Source: CAD feature listing. Evaluate the final solid. Frame: model axes, mm. A direction names the side the tool comes from. Give positions to 0.01 mm unless a question says otherwise; leave off trailing zeros. Order: outer loops, then holes, each group sorted by start corner. A loop starts at its lowest first (then second) coordinate and runs counter-clockwise, first axis right, second up. Notation, with made-up numbers: M 58.25,44.5 L 103.25,44.5 A9 ccw 103.25,57.5 Z; hole C 65,-35.5 d9. An arc over 180 degrees is marked long. Answer as a JSON object with one key per item and string values. Group by question number.
1. Section query A-A (y = -45). Output: boundary loops of the cut face in (x, z).
2. Pull-direction query (X, two-part tool) for faces 3 (the flat face through (-12.5, -1, 10)), 4 (the flat face through (-1.4, -49.2, 10)), 5 (the cylindrical face through (1.409, -51.345, 4.93)), 6 (the flat face through (-6, 1, 20)); classes: +X half, -X half, draft (parallel to the pull), parting line (faces both ways), or undercut.
3. Pin query (flat end, axial travel): P1, Ø6.5, axis at x = 1, y = -46.5, coming from the -Z side. Return the tip coordinate at first contact, or that it passes through.
4. Set-up query: faces 1 (the cylindrical face through (1.409, 38.655, 4.93)), 2 (the flat face through (-6, 1, 0)). Return all of +Z, -Z, +X, -X, +Y, -Y with unobstructed straight access to the full face (end or side cutting, diameter ignored); none if empty.
5. Section query B-B (x = 0). Output: boundary loops of the cut face in (y, z).
6. Section query C-C (z = 15.5). Output: boundary loops of the cut face in (x, y).
7. Section query D-D (y = 0). Output: boundary loops of the cut face in (x, z), plus the area to 3 significant figures.
8. Material intervals for L1, parallel to Y at x = 0, z = 5.5; L2, parallel to Y at x = 0, z = 15.75; L3, parallel to Z at x = -4.75, y = -48, sorted ascending. Write a range as [from, to].
from build123d import *

# Parameters (mm, degrees)
SKETCH1_W                   = 25
SKETCH1_H                   = 110
BOSS_EXTRUDE1_DEPTH         = 20
SKETCH3_R                   = 4.25
CUT_EXTRUDE1_DEPTH          = 30
SKETCH5_R                   = 6.5
CUT_EXTRUDE3_DEPTH          = 10
M12X1_25_TAPPED_HOLE1_D     = 10.5
M12X1_25_TAPPED_HOLE1_DEPTH = 30.25
M12X1_25_TAPPED_HOLE1_TIP   = 3.15451825


with BuildPart() as part:
    # Sketch1 → Boss-Extrude1 (new body)
    with BuildSketch(Plane.XY):
        Rectangle(SKETCH1_W, SKETCH1_H)
    extrude(amount=BOSS_EXTRUDE1_DEPTH)

    # Sketch3 → Cut-Extrude1 (cut)
    with BuildSketch(Plane.XY.offset(20)):
        with Locations((0, 45)):
            Circle(SKETCH3_R)
        with Locations((0, -45)):
            Circle(SKETCH3_R)
    extrude(amount=-CUT_EXTRUDE1_DEPTH, mode=Mode.SUBTRACT)

    # Sketch5 → Cut-Extrude3 (cut)
    with BuildSketch(Plane(origin=(0, 0, 0), x_dir=(-1, 0, 0), z_dir=(0, 0, -1))):
        with Locations((0, 45)):
            Circle(SKETCH5_R)
        with Locations((0, -45)):
            Circle(SKETCH5_R)
    extrude(amount=-CUT_EXTRUDE3_DEPTH, mode=Mode.SUBTRACT)

    # M12x1.25 Tapped Hole1
    with Locations(Plane(origin=(0, 0, 0), x_dir=(-1, 0, 0), z_dir=(0, 0, -1))):
        with Locations((0, 0)):
            Hole(M12X1_25_TAPPED_HOLE1_D / 2, depth=M12X1_25_TAPPED_HOLE1_DEPTH)
            with Locations((0, 0, -(M12X1_25_TAPPED_HOLE1_DEPTH + M12X1_25_TAPPED_HOLE1_TIP / 2))):  # 118° drill point
                Cone(0, M12X1_25_TAPPED_HOLE1_D / 2, M12X1_25_TAPPED_HOLE1_TIP, mode=Mode.SUBTRACT)


solid = part.part
Answer sheet:
{
 "1": {"outline": "M -12.5,0 L -6.5,0 L -6.5,10 L -4.25,10 L -4.25,20 L -12.5,20 Z; M 4.25,10 L 6.5,10 L 6.5,0 L 12.5,0 L 12.5,20 L 4.25,20 Z"},
 "2": {"face 3": "-X half", "face 4": "undercut", "face 5": "undercut", "face 6": "draft"},
 "3": {"P1": "z = 10"},
 "4": {"face 1": "-Z", "face 2": "-Z, +X, -X, +Y, -Y"},
 "5": {"outline": "M -55,0 L -51.5,0 L -51.5,10 L -49.25,10 L -49.25,20 L -55,20 Z; M -40.75,10 L -38.5,10 L -38.5,0 L -5.25,0 L -5.25,20 L -40.75,20 Z; M 5.25,0 L 38.5,0 L 38.5,10 L 40.75,10 L 40.75,20 L 5.25,20 Z; M 49.25,10 L 51.5,10 L 51.5,0 L 55,0 L 55,20 L 49.25,20 Z"},
 "6": {"outline": "M -12.5,-55 L 12.5,-55 L 12.5,55 L -12.5,55 Z; hole C 0,0 d10.5; hole C 0,-45 d8.5; hole C 0,45 d8.5"},
 "7": {"outline": "M -12.5,0 L -5.25,0 L -5.25,20 L -12.5,20 Z; M 5.25,0 L 12.5,0 L 12.5,20 L 5.25,20 Z", "area": "290 mm^2"},
 "8": {"L1": "[-55, -51.5], [-38.5, -5.25], [5.25, 38.5], [51.5, 55]", "L2": "[-55, -49.25], [-40.75, -5.25], [5.25, 40.75], [49.25, 55]", "L3": "[10, 20]"}
}
